```python
from build123d import *

# Parameters (mm, degrees)
BOSS_EXTRUDE1_DEPTH          = 8.2
SKETCH2_OUTSIDE_W            = 31.148
SKETCH2_OUTSIDE_H            = 28.828
SKETCH2_OUTSIDE_R            = 7.5
CUT_EXTRUDE1_DEPTH           = 8.2
CUT_EXTRUDE1_DRAFT           = -23
SKETCH3_OUTSIDE_W            = 31.148
SKETCH3_OUTSIDE_H            = 28.828
SKETCH3_OUTSIDE_R            = 7.5
CUT_EXTRUDE2_DEPTH           = 8.2
CUT_EXTRUDE2_DRAFT           = -23
M10_TAPPED_HOLE1_D           = 8.5
M10_TAPPED_HOLE1_CSINK_D     = 10.05
M10_TAPPED_HOLE1_CSINK_ANGLE = 90


with BuildPart() as part:
    # Sketch1 → Boss-Extrude1 (new body)
    with BuildSketch(Plane(origin=(0, 0, 0), x_dir=(1, 0, 0), z_dir=(0, 1, 0))):
        Polygon((4.330127019, 7.5), (-4.330127019, 7.5), (-8.660254038, 0), (-4.330127019, -7.5), (4.330127019, -7.5), (8.660254038, 0), align=None)
    extrude(amount=BOSS_EXTRUDE1_DEPTH)


with BuildPart() as cut_extrude1_tool:
    # Sketch2 outside → Cut-Extrude1 (with draft: the straight prism first)
    with BuildSketch(Plane(origin=(0, 8.2, 0), x_dir=(1, 0, 0), z_dir=(0, 1, 0))):
        Rectangle(SKETCH2_OUTSIDE_W, SKETCH2_OUTSIDE_H)
        Circle(SKETCH2_OUTSIDE_R, mode=Mode.SUBTRACT)
    extrude(amount=-CUT_EXTRUDE1_DEPTH)
    # Cut-Extrude1: the draft: its side faces are tilted about the plane it starts from
    cut_extrude1_sides = [cut_extrude1_tool.faces().sort_by_distance(p)[0] for p in [
        (0, 4.1, 14.414),
        (15.574, 4.1, 0),
        (0, 4.1, -14.414),
        (-15.574, 4.1, 0),
        (-7.5, 4.1, 0),
    ]]
    draft(cut_extrude1_sides, Plane(origin=(0, 8.2, 0), x_dir=(1, 0, 0), z_dir=(0, 1, 0)), CUT_EXTRUDE1_DRAFT)


with BuildPart() as part_1:
    add(part.part)

    # Cut-Extrude1: cut by cut_extrude1_tool
    add(cut_extrude1_tool.part, mode=Mode.SUBTRACT)


with BuildPart() as cut_extrude2_tool:
    # Sketch3 outside → Cut-Extrude2 (with draft: the straight prism first)
    with BuildSketch(Plane.XZ):
        Rectangle(SKETCH3_OUTSIDE_W, SKETCH3_OUTSIDE_H)
        Circle(SKETCH3_OUTSIDE_R, mode=Mode.SUBTRACT)
    extrude(amount=-CUT_EXTRUDE2_DEPTH)
    # Cut-Extrude2: the draft: its side faces are tilted about the plane it starts from
    cut_extrude2_sides = [cut_extrude2_tool.faces().sort_by_distance(p)[0] for p in [
        (0, 4.1, -14.414),
        (15.574, 4.1, 0),
        (0, 4.1, 14.414),
        (-15.574, 4.1, 0),
        (-7.5, 4.1, 0),
    ]]
    draft(cut_extrude2_sides, Plane.XZ, CUT_EXTRUDE2_DRAFT)


with BuildPart() as part_2:
    add(part_1.part)

    # Cut-Extrude2: cut by cut_extrude2_tool
    add(cut_extrude2_tool.part, mode=Mode.SUBTRACT)

    # M10 Tapped Hole1 (through all)
    with Locations(Plane(origin=(0, 8.2, 0), x_dir=(1, 0, 0), z_dir=(0, 1, 0))):
        with Locations((0, 0)):
            CounterSinkHole(M10_TAPPED_HOLE1_D / 2, M10_TAPPED_HOLE1_CSINK_D / 2, counter_sink_angle=M10_TAPPED_HOLE1_CSINK_ANGLE)


solid = part_2.part
```
Geometry check sheet. Reference: the model listing, model coordinates, mm. Coordinates: 2 decimals unless noted, no trailing zeros. Order: outer loops, then holes, each group sorted by start corner. A loop starts at its lowest first (then second) coordinate and runs counter-clockwise, first axis right, second up. Notation, with made-up numbers: (26, -28) - (83, -28) arc R20 cw to (83, -11) - close; hole circle Ø3 at (-38, 9.5). An arc over 180 degrees is marked (long way). Answer as a JSON object with one key per item and string values. Group by question number.
Item 1: Sectioned sample at C-C, the plane y = 7. Record the cut outline in (x, z).
Item 2: Draft check along Z on faces 1 (the face through (-2.285, 3.661, -3.584)), 2 (the face through (3.872, 7.548, 6.744)), 3 (the face through (-7.777, 0.652, 0.019)). Enter one of: +Z half, -Z half, draft (parallel to the pull), parting line (faces both ways), or undercut.
Item 3: Sectioned sample at A-A, the plane y = 4.75. Record the cut outline in (x, z), and give its area (3 significant figures).
Item 4: Sectioned sample at B-B, the plane y = 5.75. Record the cut outline in (x, z).
Item 5: Depth check by flat-ended pin: pin 1 Ø3 at (x, y) = (6, 4.5) entering from -Z; pin 2 Ø3 at (x, z) = (-4.5, -0.5) entering from +Y; pin 3 Ø1.5 at (y, z) = (1.5, 6) entering from -X; pin 4 Ø5 at (x, z) = (0, 0) entering from +Y. Enter the tip coordinate at first touch or a pass-through.
Item 6: Scan lines: probe 1 along Z at (x, y) = (0, 1.5); probe 2 along Z at (x, y) = (2.25, 2.5); probe 3 along X at (y, z) = (3.5, -2.5). Record each from-to range of solid material in increasing order.
Resolved:
{
 "1": {"outline": "(-7.9, -1.32) - (-5.09, -6.18) arc R8.01 ccw to (-2.81, -7.5) - (2.81, -7.5) arc R8.01 ccw to (5.09, -6.18) - (7.9, -1.32) arc R8.01 ccw to (7.9, 1.32) - (5.09, 6.18) arc R8.01 ccw to (2.81, 7.5) - (-2.81, 7.5) arc R8.01 ccw to (-5.09, 6.18) - (-7.9, 1.32) arc R8.01 ccw to start; hole circle Ø8.5 at (0, 0)"},
 "2": {"face 1": "undercut", "face 2": "+Z half", "face 3": "parting line"},
 "3": {"outline": "(-8.66, 0) - (-4.33, -7.5) - (4.33, -7.5) - (8.66, 0) - (4.33, 7.5) - (-4.33, 7.5) - close; hole circle Ø8.5 at (0, 0)", "area": "138 mm^2"},
 "4": {"outline": "(-8.54, -0.21) - (-4.45, -7.29) arc R8.54 ccw to (-4.08, -7.5) - (4.08, -7.5) arc R8.54 ccw to (4.45, -7.29) - (8.54, -0.21) arc R8.54 ccw to (8.54, 0.21) - (4.45, 7.29) arc R8.54 ccw to (4.08, 7.5) - (-4.08, 7.5) arc R8.54 ccw to (-4.45, 7.29) - (-8.54, 0.21) arc R8.54 ccw to start; hole circle Ø8.5 at (0, 0)"},
 "5": {"pin 1": "z = -7.21", "pin 2": "y = 8.2", "pin 3": "x = -5.63", "pin 4": "through"},
 "6": {"probe 1": "-7.5 to -4.25, 4.25 to 7.5", "probe 2": "-7.5 to -3.61, 3.61 to 7.5", "probe 3": "-7.22 to -3.44, 3.44 to 7.22"}
}
